Can you work these out from the drawing? Everything is in mm from the part's minimum corner. A direction names the side the tool comes from. Round coordinates to 2 decimals unless told otherwise and drop trailing zeros. Loops run counter-clockwise (first coordinate to the right, second up) from the corner with the lowest first, then second, coordinate; pieces in that order, holes last. Notation, with made-up numbers: (40, 65.5) - (83, 65.5) arc R20 ccw to (83, 73.5) - close; hole circle Ø1 at (69, 34). An arc over 180 degrees is marked (long way). Answer as a JSON object with one key per item and string values. Group by question number.
1) If I drill on line 1 along Y through (x, z) = (32.5, 8.75); line 2 along Y through (x, z) = (32.5, 49.5); line 3 along Z through (x, y) = (39.5, 60), over which ranges is the centre line in solid material (lowest first)? Write a range as [from, to].
2) I want a section at A-A, the plane y = 32.5. Please give me the cut outline in (x, z).
3) I want a section at B-B, the plane x = 58.5. Please give me the cut outline in (y, z).
4) Will these pins go through, and if not, where does the flat tip stop? P1, Ø1, axis at x = 28.5, z = 24.5, coming from the -Y side; P2, Ø8, axis at y = 12.5, z = 18, coming from the +X side; P3, Ø5, axis at x = 32.5, y = 58.5, coming from the +Z side; P4, Ø5, axis at x = 24.5, z = 9, coming from the +Y side.
5) Which directions (+Z, -Z, +X, -X, +Y, -Y) give clear straight access to the entire face, cutting with the end or side of a thin tool? Please do the marked faces 4 and 5.
6) If we mould it in two halves opening along X, with no side actions, what happens to the marked faces 1, 2 and 3? For each: pulls with the +X half, pulls with the -X half, needs draft (parallel to the pull), parting line crosses it, or undercut.
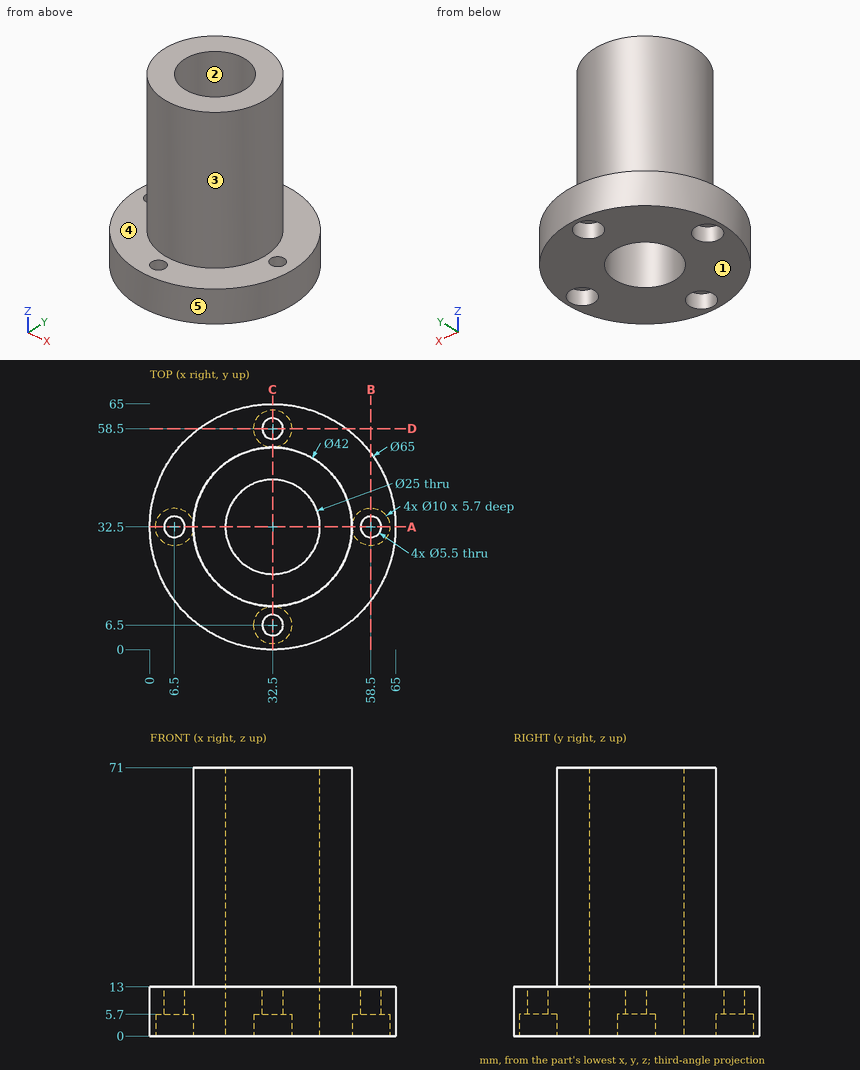
Outcome:
{
 "1": {"line 1": "[0, 3.75], [9.25, 20], [45, 55.75], [61.25, 65]", "line 2": "[11.5, 20], [45, 53.5]", "line 3": "[0, 13]"},
 "2": {"outline": "(0, 0) - (1.5, 0) - (1.5, 5.7) - (3.75, 5.7) - (3.75, 13) - (0, 13) - close; (9.25, 5.7) - (11.5, 5.7) - (11.5, 0) - (20, 0) - (20, 71) - (11.5, 71) - (11.5, 13) - (9.25, 13) - close; (45, 0) - (53.5, 0) - (53.5, 5.7) - (55.75, 5.7) - (55.75, 13) - (53.5, 13) - (53.5, 71) - (45, 71) - close; (61.25, 5.7) - (63.5, 5.7) - (63.5, 0) - (65, 0) - (65, 13) - (61.25, 13) - close"},
 "3": {"outline": "(13, 0) - (27.5, 0) - (27.5, 5.7) - (29.75, 5.7) - (29.75, 13) - (13, 13) - close; (35.25, 5.7) - (37.5, 5.7) - (37.5, 0) - (52, 0) - (52, 13) - (35.25, 13) - close"},
 "4": {"P1": "y = 11.79", "P2": "x = 46.1", "P3": "through", "P4": "y = 64.53"},
 "5": {"face 4": "+Z", "face 5": "+Z, -Z"},
 "6": {"face 1": "needs draft", "face 2": "undercut", "face 3": "parting line crosses it"}
}
